from build123d import *

# Parameters (mm, degrees)
BOSS_EXTRUDE1_DEPTH = 5.6
SKETCH2_R           = 6.35
BOSS_EXTRUDE2_DEPTH = 3.4
SKETCH3_R           = 2
BOSS_EXTRUDE3_DEPTH = 30


with BuildPart() as part:
    # Sketch1 → Boss-Extrude1 (new body)
    with BuildSketch(Plane(origin=(0, 0, 0), x_dir=(1, 0, 0), z_dir=(0, 1, 0))):
        with BuildLine():
            Line((-9.72424134, -2.15192377), (-9.725740285, -2.152789186))
            ThreePointArc((-9.725740285, -2.152789186), (-10.823817926, -6.250865027), (-6.725742085, -7.348942669))
            Line((-6.725742085, -7.348942669), (-6.723420775, -7.34760246))
            ThreePointArc((-6.723420775, -7.34760246), (-4.978167749, -8.626268935), (-2.998, -9.497952231))
            Line((-2.998, -9.497952231), (-2.998, -9.5))
            ThreePointArc((-2.998, -9.5), (0.002000003, -12.499999996), (3.002, -9.499999993))
            Line((3.002, -9.499999993), (3.002, -9.497636397))
            ThreePointArc((3.002, -9.497636397), (4.982303032, -8.625613539), (6.727581168, -7.346540363))
            Line((6.727581168, -7.346540363), (6.728741336, -7.347210186))
            ThreePointArc((6.728741336, -7.347210186), (10.826817547, -6.249133975), (9.728741336, -2.151057763))
            Line((9.728741336, -2.151057763), (9.727581168, -2.15038794))
            ThreePointArc((9.727581168, -2.15038794), (9.962651964, 0.001128196), (9.727467916, 2.152631955))
            ThreePointArc((9.727467916, 2.152631955), (10.825817547, 6.250866025), (6.727194396, 7.348626461))
            ThreePointArc((6.727194396, 7.348626461), (4.981167779, 8.628000969), (3, 9.5))
            ThreePointArc((3, 9.5), (2e-09, 12.5), (-3, 9.499052498))
            ThreePointArc((-3, 9.499052498), (-4.980665222, 8.626558938), (-6.726128008, 7.346856081))
            ThreePointArc((-6.726128008, 7.346856081), (-10.824817547, 6.249133975), (-9.726741336, 2.151057764))
            Line((-9.726741336, 2.151057764), (-9.725033927, 2.150071991))
            ThreePointArc((-9.725033927, 2.150071991), (-9.959651798, -0.000969188), (-9.72424134, -2.15192377))
        make_face()
    extrude(amount=BOSS_EXTRUDE1_DEPTH)

    # Sketch2 → Boss-Extrude2 (add)
    with BuildSketch(Plane.XZ):
        with Locations(Location((0, 0, 0), (0, 0, 90))):
            Circle(SKETCH2_R)
    extrude(amount=BOSS_EXTRUDE2_DEPTH)

    # Sketch3 → Boss-Extrude3 (add)
    with BuildSketch(Plane.XZ.offset(3.4)):
        with Locations(Location((0, 0, 0), (0, 0, 270))):
            Circle(SKETCH3_R)
    extrude(amount=BOSS_EXTRUDE3_DEPTH)


solid = part.part
Verification items for the finished model (mm, model axes). A direction names the side the tool comes from. Round coordinates to 2 decimals unless told otherwise and drop trailing zeros. Write each loop counter-clockwise with the first axis right and the second up, starting at its lowest first coordinate (ties: lowest second). Pieces come first, ordered by that corner, then holes.
(1) Mould release check, pull along Z, two halves, no side actions. Record for faces 3 (the cylindrical face through (3.86, -1.68, -5.04)), 4 (the flat face through (-2, -3.4, -2)), 5 (the cylindrical face through (10.86, 2.76, -6.19)): pulls with the +Z half, pulls with the -Z half, needs draft (parallel to the pull), parting line crosses it, or undercut.
Returned:
face 3: parting line crosses it
face 4: needs draft
face 5: undercut
(2) Section check D-D (x = 3.5). Enter the section's corners in (y, z), plus the area to 3 significant figures.
Returned:
outline: (-3.4, -5.3) - (0, -5.3) - (0, -9.33) - (5.6, -9.33) - (5.6, 9.33) - (0, 9.33) - (0, 5.3) - (-3.4, 5.3) - close
area: 140 mm2
(3) Material ranges on line 1 (Y direction, x = 8.25, z = -3.5); line 2 (Y direction, x = 0.25, z = 2.75); line 3 (Z direction, x = -0.25, y = -15), recorded low to high.
Returned:
line 1: y = 0 to 5.6
line 2: y = -3.4 to 5.6
line 3: z = -1.98 to 1.98
(4) Section check C-C (y = -23.5). Enter the section's corners in (x, z).
Returned:
outline: circle Ø4 at (0, 0)
(5) Section check A-A (z = 0). Enter the section's corners in (x, y).
Returned:
outline: (-9.96, 0) - (-6.35, 0) - (-6.35, -3.4) - (-2, -3.4) - (-2, -33.4) - (2, -33.4) - (2, -3.4) - (6.35, -3.4) - (6.35, 0) - (9.96, 0) - (9.96, 5.6) - (-9.96, 5.6) - close
(6) Depth check by flat-ended pin: pin 1 Ø8 at (x, y) = (1.5, -9.5) entering from -Z; pin 2 Ø6.5 at (x, z) = (3.5, -2) entering from -Y; pin 3 Ø3 at (y, z) = (-14, -0.5) entering from -X; pin 4 Ø12 at (y, z) = (-24, -5.5) entering from +X. Enter the tip coordinate at first touch or a pass-through.
Returned:
pin 1: stops at z = -2
pin 2: stops at y = -33.4
pin 3: stops at x = -2
pin 4: stops at x = 2
(7) Section check B-B (x = 0). Enter the section's corners in (y, z).
Returned:
outline: (-33.4, -2) - (-3.4, -2) - (-3.4, -6.35) - (0, -6.35) - (0, -12.5) - (5.6, -12.5) - (5.6, 12.5) - (0, 12.5) - (0, 6.35) - (-3.4, 6.35) - (-3.4, 2) - (-33.4, 2) - close
(8) Access from +Z, -Z, +X, -X, +Y, -Y to the whole of each face (thin tool, end or side, straight path). Record for faces 1 (the flat face through (0, 5.6, 0)), 2 (the cylindrical face through (-2, -18, 0)).
Returned:
face 1: +Z, -Z, +X, -X, +Y
face 2: -Y
